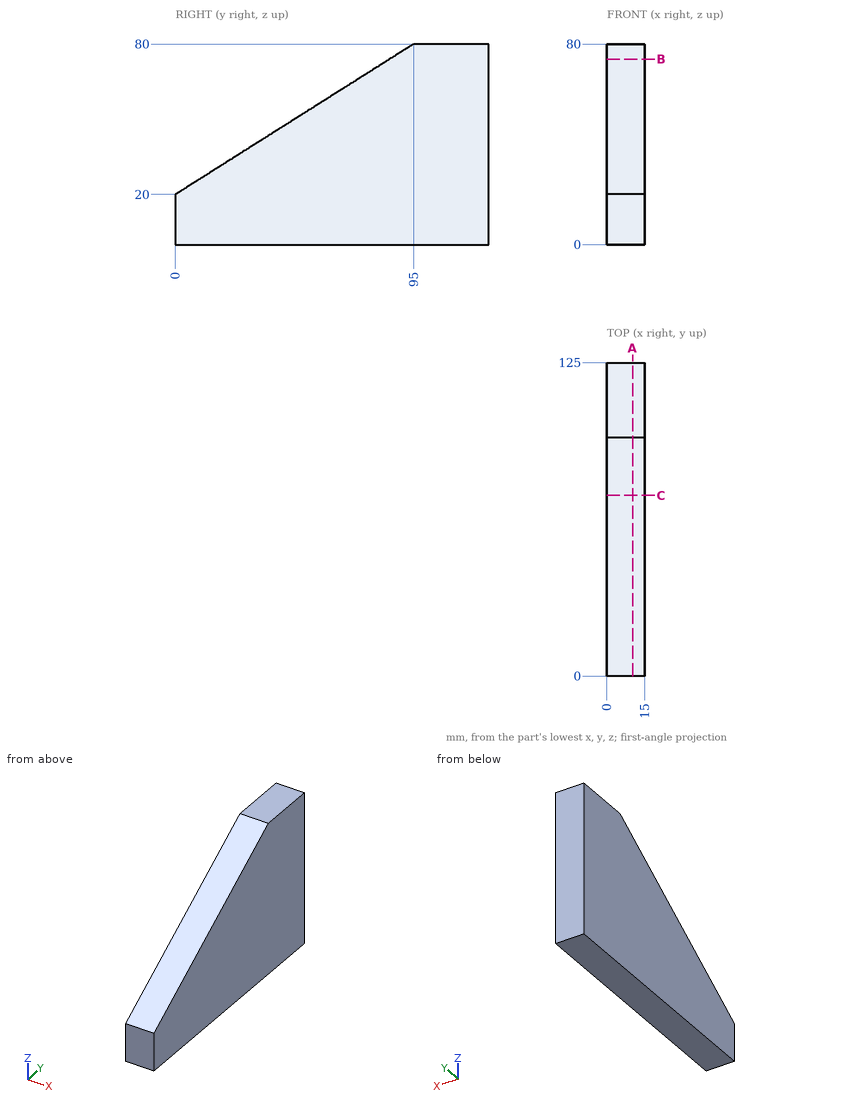
Job drawing, mm, ordinate dimensions from the low corner. One solid piece. Round coordinates to 2 decimals unless told otherwise and drop trailing zeros. Loops run counter-clockwise (first coordinate to the right, second up) from the corner with the lowest first, then second, coordinate; pieces in that order, holes last. Notation, with made-up numbers: (83.5, 12) -> (125.5, 12) arc R36 ccw to (125.5, 46) -> close; hole circle Ø11 at (-9, 4.5). An arc over 180 degrees is marked (long way). Use CSV: the item, a comma, the result in double quotes. Start each with the question number.
Q1. Saw through at A-A on x = 10.25. Give the cut face in (y, z), and give its area (3 significant figures).
Q2. Saw through at B-B on z = 74. Give the cut face in (x, y).
Q3. Drill centre lines: L1, parallel to Y at x = 9.5, z = 62.5; L2, parallel to Z at x = 10.75, y = 22; L3, parallel to Y at x = 2, z = 66.5 (3 decimals). Where is each one in solid material? Low to high.
Q4. Saw through at C-C on y = 72. Give the cut face in (x, z).
Q5. Flat gauge pin, fed straight in: pin 1 Ø3 at (x, y) = (6.5, 92.5) entering from +Z. Where does the tip first touch, or does it go through?
Solutions:
1,outline,"(0, 0) -> (125, 0) -> (125, 80) -> (95, 80) -> (0, 20) -> close"
1,area,"7,150 mm^2"
2,outline,"(0, 85.5) -> (15, 85.5) -> (15, 125) -> (0, 125) -> close"
3,L1,"y = 67.29 to 125"
3,L2,"z = 0 to 33.89"
3,L3,"y = 73.625 to 125"
4,outline,"(0, 0) -> (15, 0) -> (15, 65.47) -> (0, 65.47) -> close"
5,pin 1,"stops at z = 79.37"
